The listing builds one solid part. Answer for the finished solid, in the listing's coordinates (mm). Face numbers are marked on the shaded views. A direction names the side the tool comes from. Round coordinates to 2 decimals unless told otherwise and drop trailing zeros. Write each loop counter-clockwise with the first axis right and the second up, starting at its lowest first coordinate (ties: lowest second). Pieces come first, ordered by that corner, then holes.
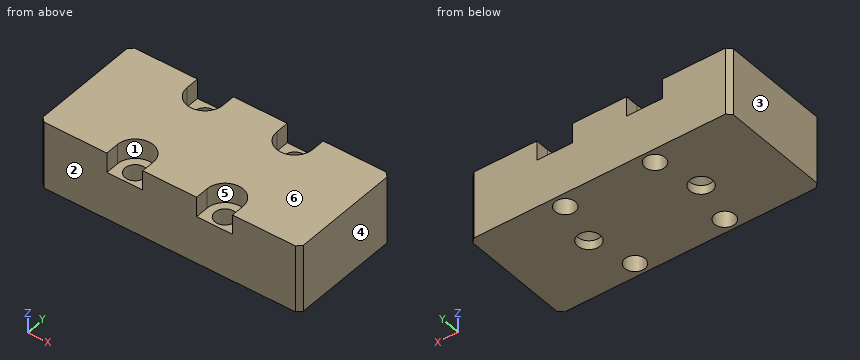
from build123d import *

# Parameters (mm, degrees)
SKETCH1_W                                           = 58
SKETCH1_H                                           = 26
BOSS_EXTRUDE1_DEPTH                                 = 7.5
CBORE_FOR_M4_HEX_SOCKET_HEAD_CAP_SCREW1_D           = 4.5
CBORE_FOR_M4_HEX_SOCKET_HEAD_CAP_SCREW1_CBORE_D     = 8
CBORE_FOR_M4_HEX_SOCKET_HEAD_CAP_SCREW1_CBORE_DEPTH = 4.4
SKETCH6_W                                           = 8
SKETCH6_H                                           = 3
CUT_EXTRUDE1_DEPTH                                  = 4.4
BLIND_PIN_HOLE1_SIZE_MM_D                           = 5
BLIND_PIN_HOLE1_SIZE_MM_DEPTH                       = 2
BLIND_PIN_HOLE1_SIZE_MM_TIP                         = 1.502151548
CHAMFER1_SIZE                                       = 1


with BuildPart() as part:
    # Sketch1 → Boss-Extrude1 (new, symmetric)
    with BuildSketch(Plane.XY):
        Rectangle(SKETCH1_W, SKETCH1_H)
    extrude(amount=BOSS_EXTRUDE1_DEPTH, both=True)

    # CBORE for M4 Hex Socket Head Cap Screw1 (through all)
    with Locations(Plane.XY.offset(7.5)):
        with Locations((-10, 10), (-10, -10), (10, -10), (10, 10)):
            CounterBoreHole(CBORE_FOR_M4_HEX_SOCKET_HEAD_CAP_SCREW1_D / 2, CBORE_FOR_M4_HEX_SOCKET_HEAD_CAP_SCREW1_CBORE_D / 2, CBORE_FOR_M4_HEX_SOCKET_HEAD_CAP_SCREW1_CBORE_DEPTH)

    # Sketch6 → Cut-Extrude1 (cut)
    with BuildSketch(Plane.XY.offset(7.5)):
        with Locations((-10, 11.5)):
            Rectangle(SKETCH6_W, SKETCH6_H)
        with Locations((10, 11.5)):
            Rectangle(SKETCH6_W, SKETCH6_H)
    cut_extrude1 = extrude(amount=-CUT_EXTRUDE1_DEPTH, mode=Mode.SUBTRACT)

    # Mirror1: Cut-Extrude1 across plane
    add(cut_extrude1.mirror(Plane.ZX), mode=Mode.SUBTRACT)

    # Blind Pin Hole1 (size mm)
    with Locations(Plane(origin=(0, 0, -7.5), x_dir=(-1, 0, 0), z_dir=(0, 0, -1))):
        with Locations((-12.5, 0), (12.5, 0)):
            Hole(BLIND_PIN_HOLE1_SIZE_MM_D / 2, depth=BLIND_PIN_HOLE1_SIZE_MM_DEPTH)
            with Locations((0, 0, -(BLIND_PIN_HOLE1_SIZE_MM_DEPTH + BLIND_PIN_HOLE1_SIZE_MM_TIP / 2))):  # 118° drill point
                Cone(0, BLIND_PIN_HOLE1_SIZE_MM_D / 2, BLIND_PIN_HOLE1_SIZE_MM_TIP, mode=Mode.SUBTRACT)

    # Chamfer1
    chamfer1_edges = [part.edges().sort_by_distance(p)[0] for p in [
        (29, -13, 0),
        (-29, -13, 0),
        (-29, 13, 0),
        (29, 13, 0),
    ]]
    chamfer(chamfer1_edges, length=CHAMFER1_SIZE)


solid = part.part
1. Section C-C on z = 5.5 is taken. Determine the outline of the cut face in (x, y).
Geometry says:
outline: (-29, -12) - (-28, -13) - (-14, -13) - (-14, -10) arc R4 cw to (-6, -10) - (-6, -13) - (6, -13) - (6, -10) arc R4 cw to (14, -10) - (14, -13) - (28, -13) - (29, -12) - (29, 12) - (28, 13) - (14, 13) - (14, 10) arc R4 cw to (6, 10) - (6, 13) - (-6, 13) - (-6, 10) arc R4 cw to (-14, 10) - (-14, 13) - (-28, 13) - (-29, 12) - close
2. A tool of negligible diameter and unlimited length cuts with its end or side. For the marked faces 1 and 2, from which of +Z, -Z, +X, -X, +Y, -Y can it reach the whole face along a straight path? Write none if from no direction.
Geometry says:
face 1: +Z, -Y
face 2: +Z, -Z, +X, -X, -Y
3. For a pull along X with two mould halves and no side action, classify the marked faces 3, 4, 5 and 6 as released by +X, released by -X, zero draft, split by the parting line, or undercut.
Geometry says:
face 3: released by -X
face 4: released by +X
face 5: undercut
face 6: zero draft
4. Given pin 1 (2 mm diameter, centred on x = -8.5, y = 10.5, fed in from +Z); pin 2 (4 mm diameter, centred on x = -12.5, y = 0, fed in from -Z), each flat-ended and moving along its own axis, determine where each tip first touches the part or whether it passes through.
Geometry says:
pin 1: stops at z = 3.1
pin 2: stops at z = -5.2
5. Section B-B on z = -2 is taken. Determine the outline of the cut face in (x, y).
Geometry says:
outline: (-29, -12) - (-28, -13) - (28, -13) - (29, -12) - (29, 12) - (28, 13) - (-28, 13) - (-29, 12) - close; hole circle Ø4.5 at (-10, -10); hole circle Ø4.5 at (-10, 10); hole circle Ø4.5 at (10, -10); hole circle Ø4.5 at (10, 10)
6. Section A-A on y = 11 is taken. Determine the outline of the cut face in (x, z).
Geometry says:
outline: (-29, -7.5) - (-12.02, -7.5) - (-12.02, 3.1) - (-14, 3.1) - (-14, 7.5) - (-29, 7.5) - close; (-7.98, -7.5) - (7.98, -7.5) - (7.98, 3.1) - (6, 3.1) - (6, 7.5) - (-6, 7.5) - (-6, 3.1) - (-7.98, 3.1) - close; (12.02, -7.5) - (29, -7.5) - (29, 7.5) - (14, 7.5) - (14, 3.1) - (12.02, 3.1) - close
7. Straight lines are drawn through the part: line 1 along X through (y, z) = (0, -6.4); line 2 along Y through (x, z) = (10, 0); line 3 along X through (y, z) = (10, 0.5). For each, find the intervals that lie inside material, in ascending order.
Geometry says:
line 1: x = -29 to -15, -10 to 10, 15 to 29
line 2: y = -13 to -12.25, -7.75 to 7.75, 12.25 to 13
line 3: x = -29 to -12.25, -7.75 to 7.75, 12.25 to 29
